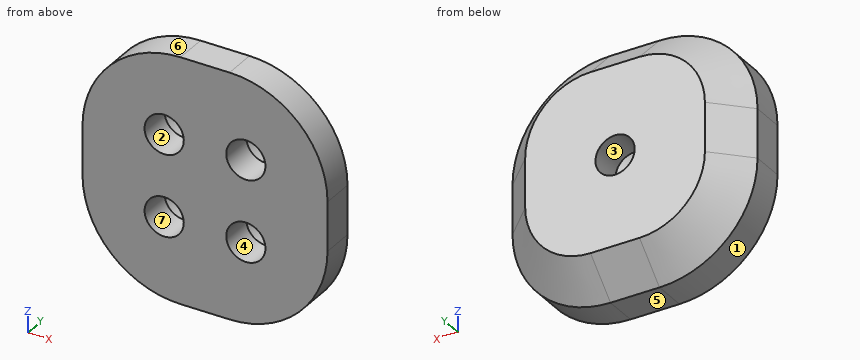
from build123d import *

# Parameters (mm, degrees)
BASE_PROFILE_SKETCH_75X75_W    = 75
BASE_PROFILE_SKETCH_75X75_H    = 75
BASE_BLOCK_75X75X20_DEPTH      = 20
CORNER_FILLETS_R30_R           = 30
TOP_EDGE_CHAMFER_10X45DEG_SIZE = 10
DOWEL_HOLE_A_12X10_D           = 12
DOWEL_HOLE_A_12X10_DEPTH       = 10
DOWEL_HOLE_A_12X10_TIP         = 3.605163714
DOWEL_HOLE_B_12X10_D           = 12
DOWEL_HOLE_B_12X10_DEPTH       = 10
DOWEL_HOLE_B_12X10_TIP         = 3.605163714


with BuildPart() as part:
    # Base Profile Sketch 75x75 → Base Block 75x75x20 (new body)
    with BuildSketch(Plane(origin=(0, 0, 0), x_dir=(1, 0, 0), z_dir=(0, 1, 0))):
        Rectangle(BASE_PROFILE_SKETCH_75X75_W, BASE_PROFILE_SKETCH_75X75_H)
    extrude(amount=BASE_BLOCK_75X75X20_DEPTH)

    # Corner Fillets R30
    corner_fillets_r30_edges = [part.edges().sort_by_distance(p)[0] for p in [
        (37.5, 10, 37.5),
        (-37.5, 10, 37.5),
        (-37.5, 10, -37.5),
        (37.5, 10, -37.5),
    ]]
    fillet(corner_fillets_r30_edges, radius=CORNER_FILLETS_R30_R)

    # Top Edge Chamfer 10x45deg
    top_edge_chamfer_10x45deg_edges = [part.edges().sort_by_distance(p)[0] for p in [
        (-37.5, 20, 0),
        (0, 20, -37.5),
        (37.5, 20, 0),
        (0, 20, 37.5),
        (-28.713203436, 20, 28.713203436),
        (28.713203436, 20, 28.713203436),
        (28.713203436, 20, -28.713203436),
        (-28.713203436, 20, -28.713203436),
    ]]
    chamfer(top_edge_chamfer_10x45deg_edges, length=TOP_EDGE_CHAMFER_10X45DEG_SIZE)

    # Dowel Hole A Ø12x10
    with Locations(Plane.ZX.offset(20)):
        with Locations((0, 0)):
            Hole(DOWEL_HOLE_A_12X10_D / 2, depth=DOWEL_HOLE_A_12X10_DEPTH)
            with Locations((0, 0, -(DOWEL_HOLE_A_12X10_DEPTH + DOWEL_HOLE_A_12X10_TIP / 2))):  # 118° drill point
                Cone(0, DOWEL_HOLE_A_12X10_D / 2, DOWEL_HOLE_A_12X10_TIP, mode=Mode.SUBTRACT)

    # Dowel Hole B Ø12x10
    with Locations(Plane(origin=(-12.5, 0, 12.5), x_dir=(0, 0, -1), z_dir=(0, -1, 0))):
        with Locations((0, 0), (0, 25), (25, 25), (25, 0)):
            Hole(DOWEL_HOLE_B_12X10_D / 2, depth=DOWEL_HOLE_B_12X10_DEPTH)
            with Locations((0, 0, -(DOWEL_HOLE_B_12X10_DEPTH + DOWEL_HOLE_B_12X10_TIP / 2))):  # 118° drill point
                Cone(0, DOWEL_HOLE_B_12X10_D / 2, DOWEL_HOLE_B_12X10_TIP, mode=Mode.SUBTRACT)


solid = part.part
Check sheet for the modelled part. Datum: model origin and axes. Units: mm. Face numbers are marked on the shaded views. A direction names the side the tool comes from. Coordinates: 2 decimals unless noted, no trailing zeros. Loops run counter-clockwise (first coordinate to the right, second up) from the corner with the lowest first, then second, coordinate; pieces in that order, holes last. Notation, with made-up numbers: (26, -6.75) -> (67, -6.75) arc R24 ccw to (67, 23.25) -> close; hole circle Ø3 at (4.5, 14.25). An arc over 180 degrees is marked (long way). Write item = value, one per line. Start each with the question number.
1. Depth check by flat-ended pin: P1, Ø1, axis at x = -17.5, y = 11, coming from the -Z side; P2, Ø1.5, axis at y = 15, z = -6.5, coming from the -X side; P3, Ø2, axis at x = -18, y = 3.5, coming from the +Z side. Enter the tip coordinate at first touch or a pass-through.
2. Tool access check on the marked faces 1, 2 and 3. Record the directions out of +Z, -Z, +X, -X, +Y, -Y that give a thin tool (end or side, any length) a straight path to the whole face; none if there is none.
3. Section check A-A on y = 15.5. Record the cut outline in (x, z).
4. Material ranges on line 1 (Z direction, x = -12.5, y = 5.5); line 2 (X direction, y = 8, z = -15), recorded low to high.
5. Draft check along Z on the marked faces 4, 5, 6 and 7. Enter one of: released by +Z, released by -Z, zero draft, split by the parting line, or undercut.
Responses:
q1.P1 = -35.28
q1.P2 = -33.25
q1.P3 = 35.96
q2.face_1 = -Z, -X, +Y, -Y
q2.face_2 = -Y
q2.face_3 = +Y
q3.outline = (-32, -7.5) arc R24.5 ccw to (-7.5, -32) -> (7.5, -32) arc R24.5 ccw to (32, -7.5) -> (32, 7.5) arc R24.5 ccw to (7.5, 32) -> (-7.5, 32) arc R24.5 ccw to (-32, 7.5) -> close; hole circle Ø12 at (0, 0)
q4.line_1 = -37.08 to -18.5, -6.5 to 6.5, 18.5 to 37.08
q4.line_2 = -36.55 to -17.95, -7.05 to 7.05, 17.95 to 36.55
q5.face_4 = undercut
q5.face_5 = released by -Z
q5.face_6 = released by +Z
q5.face_7 = undercut
